Answer from the drawing. Dimensions are ordinates in mm from the lowest x, y and z of the part. Give positions to 0.01 mm unless a question says otherwise; leave off trailing zeros. Loops run counter-clockwise (first coordinate to the right, second up) from the corner with the lowest first, then second, coordinate; pieces in that order, holes last.
(1) Find section C-C, the plane z = 10.5. Write down the section's boundary in (x, y), then the cut area to 3 significant figures.
(2) Straight lines are drawn through the part: probe 1 along Y at (x, z) = (25, 8.25); probe 2 along X at (y, z) = (33, 2); probe 3 along X at (y, z) = (36.5, 15.75). For each, find the intervals that lie inside material, in ascending order.
(3) Each of these flat-tipped pins is pushed along its axis until it touches: P1, Ø5, axis at y = 32.5, z = 5.5, coming from the -X side; P2, Ø8, axis at x = 29.5, z = 4.5, coming from the +Y side (3 decimals); P3, Ø1.5, axis at y = 15.5, z = 5, coming from the +X side; P4, Ø24, axis at x = 25, y = 25, coming from the -Z side. Where does it stop, or does it pass through?
(4) Determine the mould class of the marked faces 1, 2 and 3 for opening direction X: pulls with the +X half, pulls with the -X half, needs draft (parallel to the pull), parting line crosses it, or undercut.
(5) Find section A-A, the plane y = 25. Write down the section's boundary in (x, z).
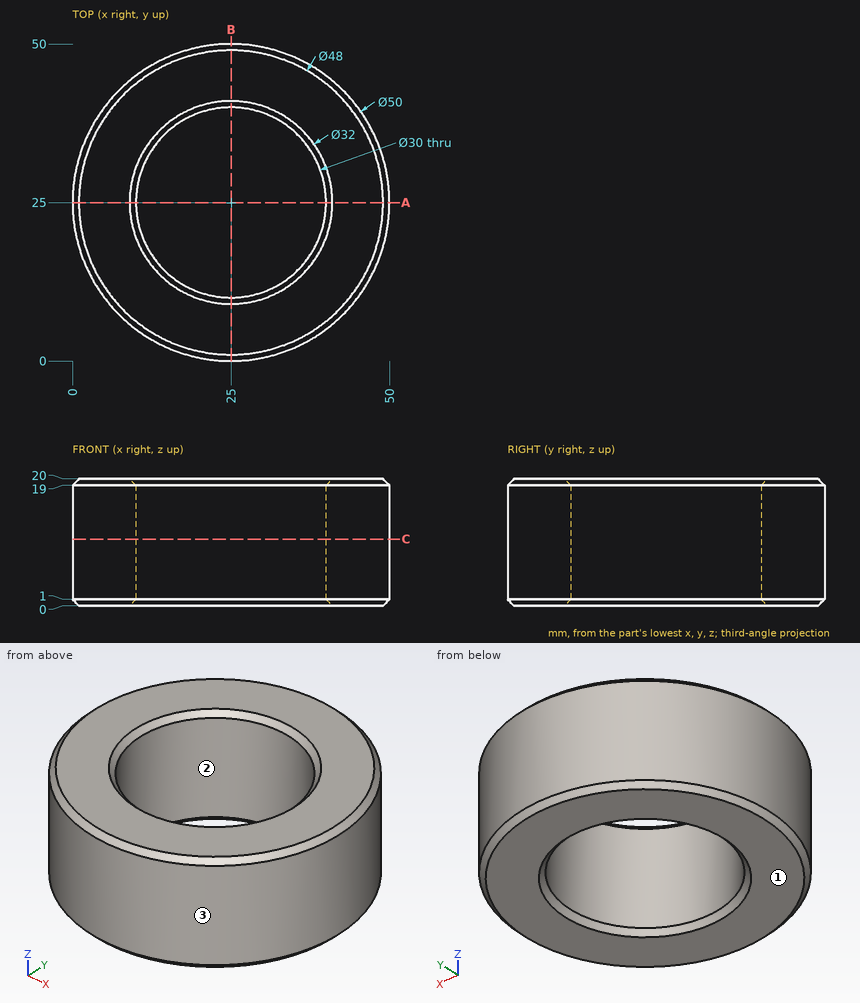
Entries:
1. outline: circle Ø50 at (25, 25); hole circle Ø30 at (25, 25)
1. area: 1,260 mm2
2. probe 1: y = 0 to 10, 40 to 50
2. probe 2: x = 1.31 to 12.31, 37.69 to 48.69
2. probe 3: x = 2.8 to 15.37, 34.63 to 47.2
3. P1: stops at x = 0.51
3. P2: stops at y = 49.995
3. P3: stops at x = 48.42
3. P4: passes through
4. face 1: needs draft
4. face 2: undercut
4. face 3: parting line crosses it
5. outline: (0, 1) - (1, 0) - (9, 0) - (10, 1) - (10, 19) - (9, 20) - (1, 20) - (0, 19) - close; (40, 1) - (41, 0) - (49, 0) - (50, 1) - (50, 19) - (49, 20) - (41, 20) - (40, 19) - close
